Build history of the part. All positions in model axes, mm. Face numbers are marked on the shaded views. Give positions to 0.01 mm unless a question says otherwise; leave off trailing zeros. Order: outer loops, then holes, each group sorted by start corner. A loop starts at its lowest first (then second) coordinate and runs counter-clockwise, first axis right, second up. Notation, with made-up numbers: (76.5, 21) - (98.5, 21) arc R15 cw to (98.5, 35) - close; hole circle Ø9 at (-29.75, -27). An arc over 180 degrees is marked (long way). Write each question's results on one line, items separated by ' | '. Start each with the question number.
1) Cut at C-C on z = -15. List the corners of the cut face in (x, y), plus the area to 3 significant figures.
2) Cut at D-D on z = -3. List the corners of the cut face in (x, y).
3) Two-plate mould, pull along Y, no slides. Class the marked faces 1 and 2: +Y half, -Y half, draft (parallel to the pull), parting line (faces both ways), or undercut.
4) Drill centre lines: line 1 along Y through (x, z) = (0, -20.5); line 2 along X through (y, z) = (7, -32.5); line 3 along Y through (x, z) = (-16, -11). Where is each one in solid material? Low to high. Write a range as from..to.
5) Drop flat-ended pins along their axis: pin 1 Ø1 at (x, z) = (-12.5, -12) entering from +Y; pin 2 Ø5 at (y, z) = (0.5, -5.5) entering from -X; pin 3 Ø10 at (x, z) = (-7.5, -12.5) entering from +Y; pin 4 Ø6 at (x, y) = (3, 16) entering from +Z. Give the stop position or say it passes through.
from build123d import *

# Parameters (mm, degrees)
CUT_EXTRUDE1_START = -10
SKETCH2_R          = 21.35
SKETCH2_R_2        = 21.34
CUT_EXTRUDE1_DEPTH = 10


with BuildPart() as part:
    # Sketch1 → Revolve-Thin1 (revolve)
    with BuildSketch(Plane(origin=(0, 0, 0), x_dir=(0, 0, -1), z_dir=(1, 0, 0)), mode=Mode.PRIVATE) as revolve_thin1_sk:
        with BuildLine():
            Line((0, 21.35), (27.854248689, 21.35))
            ThreePointArc((27.854248689, 21.35), (28.56135547, 21.479171307), (29.177124344, 21.85))
            ThreePointArc((29.177124344, 21.85), (30.5, 22.35), (31.822875656, 21.85))
            ThreePointArc((31.822875656, 21.85), (32.43864453, 21.479171307), (33.145751311, 21.35))
            Line((33.145751311, 21.35), (35, 21.35))
            Line((35, 21.35), (35, 19.75))
            Line((35, 19.75), (33.145751311, 19.75))
            ThreePointArc((33.145751311, 19.75), (31.872959105, 19.982508352), (30.764575131, 20.65))
            ThreePointArc((30.764575131, 20.65), (30.5, 20.75), (30.235424869, 20.65))
            ThreePointArc((30.235424869, 20.65), (29.127040895, 19.982508352), (27.854248689, 19.75))
            Line((27.854248689, 19.75), (0, 19.75))
            Line((0, 19.75), (0, 21.35))
        make_face()
    revolve(revolve_thin1_sk.sketch.rotate(Axis((0, 0, 0), (0, 0, -1)), 90), axis=Axis((0, 0, 0), (0, 0, -1)))

    # Sketch2 → Cut-Extrude1 (cut)
    with BuildSketch(Plane.XY.offset(CUT_EXTRUDE1_START)):
        Circle(SKETCH2_R)
        Circle(SKETCH2_R_2, mode=Mode.SUBTRACT)
    extrude(amount=CUT_EXTRUDE1_DEPTH, mode=Mode.SUBTRACT)


solid = part.part
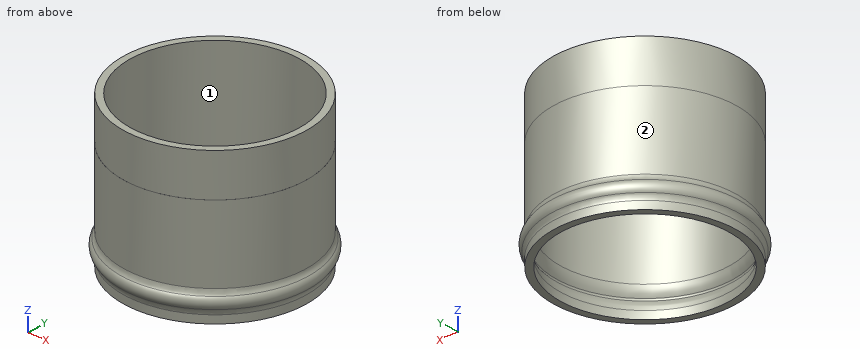
Results:
1) outline: circle Ø42.7 at (0, 0); hole circle Ø39.5 at (0, 0) | area: 207 mm^2
2) outline: circle Ø42.68 at (0, 0); hole circle Ø39.5 at (0, 0)
3) face 1: undercut | face 2: parting line
4) line 1: -21.35..-19.75, 19.75..21.35 | line 2: -20.28..-18.53, 18.53..20.28 | line 3: -14.14..-11.58, 11.58..14.14
5) pin 1: y = 17.66 | pin 2: x = -21.34 | pin 3: y = 21.2 | pin 4: through
